Can you work these out from the model? Positions are in its coordinate system, mm. A direction names the side the tool comes from. Give positions to 0.01 mm unless a question says otherwise; leave off trailing zeros. Write each loop counter-clockwise with the first axis right and the second up, starting at its lowest first coordinate (ties: lowest second). Pieces come first, ordered by that corner, then holes. Notation, with made-up numbers: M 7.5,14 L 32.5,14 A24 cw 32.5,28 Z; hole C 88,84.5 d7. An arc over 180 degrees is marked long. Answer as CSV lines item,"result". Start each with the question number.
```python
from build123d import *

# Parameters (mm, degrees)
HUB_BLOCK_SKETCH_W = 35
HUB_BLOCK_SKETCH_H = 15
HUB_BLOCK_DEPTH    = 12
DRIVE_TAB_SKETCH_W = 6
DRIVE_TAB_SKETCH_H = 4
DRIVE_TAB_DEPTH    = 5.5
SHAFT_SKETCH_R     = 4
SHAFT_8_DEPTH      = 75
PIN_HOLE_SKETCH_R  = 2
PIN_HOLE_4_DEPTH   = 75


with BuildPart() as part:
    # Hub Block Sketch → Hub Block (new body)
    with BuildSketch(Plane.XY):
        Rectangle(HUB_BLOCK_SKETCH_W, HUB_BLOCK_SKETCH_H)
    extrude(amount=HUB_BLOCK_DEPTH)

    # Drive Tab Sketch → Drive Tab (add)
    with BuildSketch(Plane.ZY.offset(17.5)):
        with Locations((6, -5.5)):
            Rectangle(DRIVE_TAB_SKETCH_W, DRIVE_TAB_SKETCH_H)
    extrude(amount=DRIVE_TAB_DEPTH)

    # Shaft Sketch → Shaft Ø8 (add)
    with BuildSketch(Plane(origin=(17.5, 0, 0), x_dir=(0, 0, -1), z_dir=(1, 0, 0))):
        with Locations((-6, 0)):
            Circle(SHAFT_SKETCH_R)
    extrude(amount=SHAFT_8_DEPTH)

    # Ball Knob Sketch → Ball Knob Ø30 (revolve)
    with BuildSketch(Plane(origin=(0, 0, 0), x_dir=(1, 0, 0), z_dir=(0, 1, 0))):
        with BuildLine():
            Line((92.5, 9), (92.5, -21))
            ThreePointArc((92.5, -21), (107.5, -6), (92.5, 9))
        make_face()
    revolve(axis=Axis((92.5, 0, 0), (0, 0, 1)))

    # Pin Hole Sketch → Pin Hole Ø4 (cut)
    with BuildSketch(Plane.XY.offset(12)):
        with Locations((-3.5, 0)):
            Circle(PIN_HOLE_SKETCH_R)
    extrude(amount=-PIN_HOLE_4_DEPTH, mode=Mode.SUBTRACT)


solid = part.part
```
1) I want a section at D-D, the plane y = 0. Please give me the cut outline in (x, z).
2) I want a section at A-A, the plane y = -6.25. Please give me the cut outline in (x, z), then the cut area to 3 significant figures.
3) I'm going to push flat-ended pins straight in: P1, Ø6, axis at y = -0.5, z = -1.5, coming from the +X side; P2, Ø16.5, axis at x = 7.5, y = 0, coming from the +Z side; P3, Ø3, axis at x = -20.5, z = 5, coming from the +Y side. Where does each tip first touch, or does it pass through?
4) I need wall thicknesses on L1, parallel to Y at x = -3.5, z = 9.5; L2, parallel to Y at x = -7.5, z = 10.5; L3, parallel to Y at x = -5, z = 11.5. Which ranges of each line are inside material? Lowest first, please. Write a range as from..to.
5) On a 3-axis mill with a long thin cutter (end or side, diameter ignored), from which of +Z, -Z, +X, -X, +Y, -Y can I reach the whole of each face in a straight line? I mean faces 1 (the flat face through (-20, -3.5, 6)), 2 (the flat face through (-20, -6, 9)), 3 (the flat face through (-3, -7.5, 6)), 4 (the flat face through (17.5, -3, 3)). Say none if no direction works.
6) Thinking about a two-plate mould opening in X: for faces 5 (the cylindrical face through (-5.1, -1.2, 6.1)), 6 (the flat face through (-23, -5, 6)), 7 (the flat face through (-20, -6, 3)), which applies, released by +X, released by -X, zero draft, split by the parting line, or undercut?
7) I want a section at B-B, the plane x = -3.5. Please give me the cut outline in (y, z), then the cut area to 3 significant figures.
8) I want a section at C-C, the plane z = 6. Please give me the cut outline in (x, y), then the cut area to 3 significant figures.
Values found:
1,outline,"M -17.5,0 L -5.5,0 L -5.5,12 L -17.5,12 Z; M -1.5,0 L 17.5,0 L 17.5,2 L 78.04,2 A15 ccw long 78.04,10 L 17.5,10 L 17.5,12 L -1.5,12 Z"
2,outline,"M -23,3 L -17.5,3 L -17.5,0 L 17.5,0 L 17.5,12 L -17.5,12 L -17.5,9 L -23,9 Z; C 92.5,6 d27.27"
2,area,"1,040 mm²"
3,P1,"stops at x = 106.8"
3,P2,"stops at z = 12"
3,P3,"stops at y = -3.5"
4,L1,"y = -7.5..-2, 2..7.5"
4,L2,"y = -7.5..7.5"
4,L3,"y = -7.5..-1.32, 1.32..7.5"
5,face 1,"+Z, -Z, -X, +Y"
5,face 2,"+Z, -X, +Y, -Y"
5,face 3,"+Z, -Z, -X, -Y"
5,face 4,"none"
6,face 5,"undercut"
6,face 6,"released by -X"
6,face 7,"zero draft"
7,outline,"M -7.5,0 L -2,0 L -2,12 L -7.5,12 Z; M 2,0 L 7.5,0 L 7.5,12 L 2,12 Z"
7,area,"132 mm²"
8,outline,"M -23,-7.5 L 17.5,-7.5 L 17.5,-4 L 78.04,-4 A15 ccw long 78.04,4 L 17.5,4 L 17.5,7.5 L -17.5,7.5 L -17.5,-3.5 L -23,-3.5 Z; hole C -3.5,0 d4"
8,area,"1,720 mm²"
